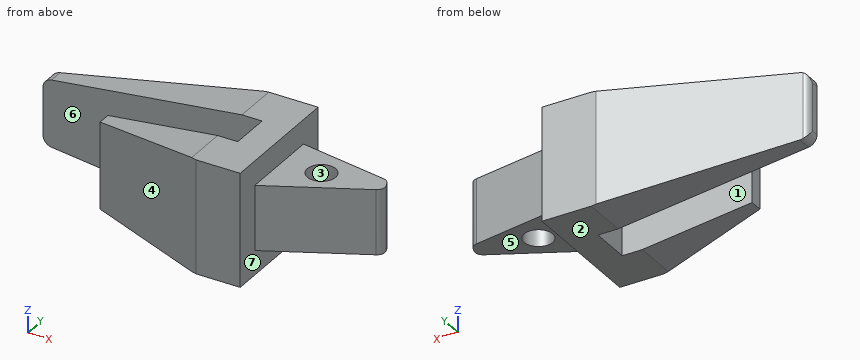
from build123d import *

# Parameters (mm, degrees)
BOSS_EXTRUDE1_DEPTH      = 80
CUT_EXTRUDE1_DEPTH       = 177.164695669
CUT_EXTRUDE1_DEPTH_BACK  = 177.164695669
SKETCH2_OUTSIDE_W        = 192.26
SKETCH2_OUTSIDE_H        = 119.26
BOSS_EXTRUDE2_DEPTH      = 20
BOSS_EXTRUDE2_DEPTH_BACK = 20
M20_TAPPED_HOLE1_D       = 17.5


with BuildPart() as part:
    # Sketch1 → Boss-Extrude1 (new body)
    with BuildSketch(Plane(origin=(0, 0, 0), x_dir=(1, 0, 0), z_dir=(0, 1, 0))):
        with BuildLine():
            Line((0, 14.689353522), (0, -14.689353522))
            ThreePointArc((0, -14.689353522), (1.507118597, -18.666037655), (5.271338899, -20.644943585))
            Line((5.271338899, -20.644943585), (122.6, -35))
            Line((122.6, -35), (153, -35))
            Line((153, -35), (153, 35))
            Line((153, 35), (122.6, 35))
            Line((122.6, 35), (5.271338899, 20.644943585))
            ThreePointArc((5.271338899, 20.644943585), (1.507118597, 18.666037655), (0, 14.689353522))
        make_face()
    extrude(amount=BOSS_EXTRUDE1_DEPTH)

    # Sketch2 outside → Cut-Extrude1 (cut, two sides: drawn at the far end of the back side and taken through both)
    with BuildSketch(Plane.XY.offset(-CUT_EXTRUDE1_DEPTH_BACK)):
        with Locations((76.5, 40)):
            Rectangle(SKETCH2_OUTSIDE_W, SKETCH2_OUTSIDE_H)
        with BuildLine():
            Line((153, 80), (153, 0))
            Line((153, 0), (125.9, 0))
            Line((125.9, 0), (55, 19.5))
            Line((55, 19.5), (55, 27.5))
            Line((55, 27.5), (135, 27.5))
            Line((135, 27.5), (135, 52.5))
            Line((135, 52.5), (0, 52.5))
            Line((0, 52.5), (0, 57.099356274))
            ThreePointArc((0, 57.099356274), (0.95248476, 59.69023467), (3.35632543, 61.047226972))
            Line((3.35632543, 61.047226972), (119.6, 80))
            Line((119.6, 80), (153, 80))
        make_face(mode=Mode.SUBTRACT)
    extrude(amount=CUT_EXTRUDE1_DEPTH + CUT_EXTRUDE1_DEPTH_BACK, mode=Mode.SUBTRACT)

    # Sketch3 → Boss-Extrude2 (add, two sides: drawn at the far end of the back side and taken through both)
    with BuildSketch(Plane.XY.offset(-BOSS_EXTRUDE2_DEPTH_BACK)):
        with BuildLine():
            Line((153, 65), (153, 15))
            Line((153, 15), (210.269952499, 44.180498289))
            ThreePointArc((210.269952499, 44.180498289), (212.69221031, 46.908347535), (212.616617933, 50.555645193))
            Line((212.616617933, 50.555645193), (211.637866551, 52.908901571))
            ThreePointArc((211.637866551, 52.908901571), (210.127565677, 54.906796263), (207.837878429, 55.921648096))
            Line((207.837878429, 55.921648096), (153, 65))
        make_face()
    extrude(amount=BOSS_EXTRUDE2_DEPTH + BOSS_EXTRUDE2_DEPTH_BACK)

    # M20 Tapped Hole1 (through all)
    with Locations(Plane.XY.offset(20)):
        with Locations((176.6, 44.2)):
            Hole(M20_TAPPED_HOLE1_D / 2)


solid = part.part
The listing builds one solid part. Answer for the finished solid, in the listing's coordinates (mm). Face numbers are marked on the shaded views. A direction names the side the tool comes from. Coordinates: 2 decimals unless noted, no trailing zeros. Order: outer loops, then holes, each group sorted by start corner. A loop starts at its lowest first (then second) coordinate and runs counter-clockwise, first axis right, second up.
Q1. A cutting plane is placed at C-C, the plane y = 38. Write down the section's boundary in (x, z), and give its area (3 significant figures).
Q2. A cutting plane is placed at D-D, the plane z = -24.5. Write down the section's boundary in (x, y).
Q3. Consider line 1 (Y direction, x = 82, z = -4.5); line 2 (Z direction, x = 162, y = 41); line 3 (Y direction, x = 176.6, z = -7.5). Determine where each line is inside the solid, lowest interval first.
Q4. Which of the six approach directions +Z, -Z, +X, -X, +Y, -Y give full straight-line access (tool end or side, diameter ignored) to the marked faces 5, 6 and 7?
Q5. A cutting plane is placed at B-B, the plane x = 176.6. Write down the section's boundary in (y, z).
Q6. A cutting plane is placed at A-A, the plane z = -5. Write down the section's boundary in (x, y).
Q7. For a pull along Y with two mould halves and no side action, classify the marked faces 1, 2, 3 and 4 as pulls with the +Y half, pulls with the -Y half, needs draft (parallel to the pull), parting line crosses it, or undercut.
Q8. Given P1, Ø15, axis at x = 191, y = 47, coming from the +Z side; P2, Ø20, axis at x = 176.6, y = 44.2, coming from the -Z side; P3, Ø20, axis at y = 35, z = 2.5, coming from the -X side; P4, Ø21, axis at y = 49, z = 10, coming from the +X side, each flat-ended and moving along its own axis, determine where each tip first touches the part or whether it passes through.
Answers follow:
1. outline: (135, -35) - (153, -35) - (153, -20) - (170.43, -20) - (170.43, 20) - (153, 20) - (153, 35) - (135, 35) - close; (182.77, -20) - (198.14, -20) - (198.14, 20) - (182.77, 20) - close
1. area: 2,570 mm2
2. outline: (36.78, 52.5) - (135, 52.5) - (135, 27.5) - (55, 27.5) - (55, 19.5) - (125.9, 0) - (153, 0) - (153, 80) - (119.6, 80) - (36.78, 66.5) - close
3. line 1: y = 12.07 to 27.5, 52.5 to 73.87
3. line 2: z = -20 to 20
3. line 3: y = 27.02 to 35.45, 52.95 to 61.09
4. face 5: -Z, +X, +Y, -Y
4. face 6: +Z, -Z, -X
4. face 7: +X
5. outline: (27.02, -20) - (35.45, -20) - (35.45, 20) - (27.02, 20) - close; (52.95, -20) - (61.09, -20) - (61.09, 20) - (52.95, 20) - close
6. outline: (0, 52.5) - (135, 52.5) - (135, 27.5) - (55, 27.5) - (55, 19.5) - (125.9, 0) - (153, 0) - (153, 15) - (210.27, 44.18) arc R5 ccw to (212.62, 50.56) - (211.64, 52.91) arc R5 ccw to (207.84, 55.92) - (153, 65) - (153, 80) - (119.6, 80) - (3.36, 61.05) arc R4 ccw to (0, 57.1) - close; hole circle Ø17.5 at (176.6, 44.2)
7. face 1: undercut
7. face 2: needs draft
7. face 3: undercut
7. face 4: pulls with the -Y half
8. P1: stops at z = 20
8. P2: stops at z = -20
8. P3: stops at x = 55
8. P4: stops at x = 213
